Verification items for the finished model (mm, model axes). Round coordinates to 2 decimals unless told otherwise and drop trailing zeros. Write each loop counter-clockwise with the first axis right and the second up, starting at its lowest first coordinate (ties: lowest second). Pieces come first, ordered by that corner, then holes.
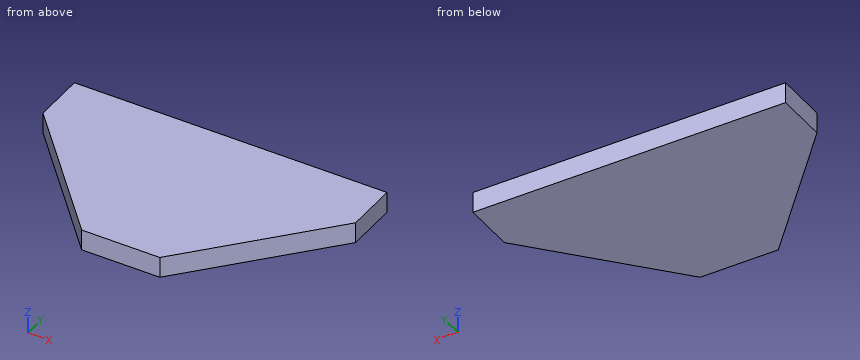
from build123d import *

# Parameters (mm, degrees)
SKETCH1_W           = 120
SKETCH1_H           = 70
BOSS_EXTRUDE1_DEPTH = 8
CUT_EXTRUDE1_DEPTH  = 8


with BuildPart() as part:
    # Sketch1 → Boss-Extrude1 (new body)
    with BuildSketch(Plane.XY):
        Rectangle(SKETCH1_W, SKETCH1_H)
    extrude(amount=BOSS_EXTRUDE1_DEPTH)

    # Sketch2 → Cut-Extrude1 (cut)
    with BuildSketch(Plane.XY.offset(8)):
        Polygon((-60, 15), (-15, -35), (-60, -35), align=None)
        Polygon((15, -35), (60, 15), (60, -35), align=None)
    extrude(amount=-CUT_EXTRUDE1_DEPTH, mode=Mode.SUBTRACT)


solid = part.part
Q1. Material ranges on line 1 along X through (y, z) = (4.5, 4.75); line 2 along Y through (x, z) = (-22.5, 6.25); line 3 along X through (y, z) = (-29, 4), recorded low to high.
Recorded:
line 1: x = -50.55 to 50.55
line 2: y = -26.67 to 35
line 3: x = -20.4 to 20.4
Q2. Sectioned sample at A-A (z = 4.25). Enter the section's corners in (x, y), plus the area to 3 significant figures.
Recorded:
outline: (-60, 15) - (-15, -35) - (15, -35) - (60, 15) - (60, 35) - (-60, 35) - close
area: 6,150 mm2
Q3. Depth check by flat-ended pin: P1, Ø3, axis at x = 18.5, z = 1.5, coming from the -Y side; P2, Ø1, axis at y = -27, z = 6, coming from the +X side; P3, Ø2, axis at y = 12, z = 2, coming from the -X side. Enter the tip coordinate at first touch or a pass-through.
Recorded:
P1: stops at y = -32.78
P2: stops at x = 22.65
P3: stops at x = -58.2
Q4. Sectioned sample at B-B (y = 10.5). Enter the section's corners in (x, z).
Recorded:
outline: (-55.95, 0) - (55.95, 0) - (55.95, 8) - (-55.95, 8) - close
Q5. Sectioned sample at C-C (x = -35.5). Enter the section's corners in (y, z).
Recorded:
outline: (-12.22, 0) - (35, 0) - (35, 8) - (-12.22, 8) - close
